Check sheet for the modelled part. Datum: model origin and axes. Units: mm. A direction names the side the tool comes from. Give positions to 0.01 mm unless a question says otherwise; leave off trailing zeros. Order: outer loops, then holes, each group sorted by start corner. A loop starts at its lowest first (then second) coordinate and runs counter-clockwise, first axis right, second up.
Item 1: Sectioned sample at D-D on y = 24. Record the boundary of the cut face in (x, z), and give its area (3 significant figures).
Item 2: Sectioned sample at B-B on x = 0. Record the boundary of the cut face in (y, z).
Item 3: Release check for a two-part mould opening along Z. For faces 1 (the cylindrical face through (-45.72, 22.32, -45.49)), 2 (the flat face through (44, 22, 0)), 3 (the flat face through (45, 35, 0)) record: released by +Z, released by -Z, zero draft, split by the parting line, or undercut.
Item 4: Sectioned sample at C-C on z = 17.5. Record the boundary of the cut face in (x, y).
Item 5: Sectioned sample at A-A on y = -3. Count the separate pieces of the cut face and the enclosed holes in it, and give its area (3 significant figures).
Item 6: Access from +Z, -Z, +X, -X, +Y, -Y to the whole of each face (thin tool, end or side, straight path). Record for faces 4 (the flat face through (73, -10, 6)), 5 (the flat face through (84.064, 0.14, 39.556)), 6 (the cylindrical face through (41.434, 22.325, -41.294)), 7 (the cylindrical face through (45.49, 22.32, -45.72)).
Item 7: Material ranges on line 1 along X through (y, z) = (2, -65); line 2 along X through (y, z) = (-7.8, 0); line 3 along Z through (x, y) = (-22, 26), recorded low to high.
Item 8: Gauge pin test, flat ends, axial feed: P1, Ø4, axis at y = 13, z = -57, coming from the +X side; P2, Ø6, axis at x = -65.5, z = 20.5, coming from the +Y side; P3, Ø1, axis at y = 20.5, z = 19.5, coming from the -X side; P4, Ø1.5, axis at x = 62.5, z = 17.5, coming from the -Y side. Record the tip position at first contact, or that the pin passes through.
from build123d import *

# Parameters (mm, degrees)
BASE_FLANGE_SKETCH_R      = 6.5
BASE_FLANGE_DEPTH         = 10
SQUARE_BOSS_DEPTH         = 25
BOSS_POCKET_DEPTH         = 130.711217711
BOSS_POCKET_DEPTH_BACK    = 130.711217711
BOSS_POCKET_SKETCH_R      = 9.473120825
RECESS_CUT_3MM_DEPTH      = 136
RECESS_CUT_3MM_DEPTH_BACK = 3
RECESS_SKETCH_R           = 72.5
RECESS_SKETCH_R_2         = 52.5


with BuildPart() as part:
    # Base Flange Sketch → Base Flange (new, symmetric)
    with BuildSketch(Plane(origin=(0, 0, 0), x_dir=(1, 0, 0), z_dir=(0, 1, 0))):
        with BuildLine():
            Line((-89.148145657, 58.529523872), (-78.836109635, 20.044481509))
            ThreePointArc((-78.836109635, 20.044481509), (-78.436026062, 17.398303615), (-78.632364827, 14.72926345))
            ThreePointArc((-78.632364827, 14.72926345), (-80, 0), (-78.632364827, -14.72926345))
            ThreePointArc((-78.632364827, -14.72926345), (-78.436026062, -17.398303615), (-78.836109635, -20.044481509))
            Line((-78.836109635, -20.044481509), (-89.148145657, -58.529523872))
            ThreePointArc((-89.148145657, -58.529523872), (-82.67766953, -82.67766953), (-58.529523872, -89.148145657))
            Line((-58.529523872, -89.148145657), (-20.044481509, -78.836109635))
            ThreePointArc((-20.044481509, -78.836109635), (-17.398303615, -78.436026062), (-14.72926345, -78.632364827))
            ThreePointArc((-14.72926345, -78.632364827), (0, -80), (14.72926345, -78.632364827))
            ThreePointArc((14.72926345, -78.632364827), (17.398303615, -78.436026062), (20.044481509, -78.836109635))
            Line((20.044481509, -78.836109635), (58.529523872, -89.148145657))
            ThreePointArc((58.529523872, -89.148145657), (82.67766953, -82.67766953), (89.148145657, -58.529523872))
            Line((89.148145657, -58.529523872), (78.836109635, -20.044481509))
            ThreePointArc((78.836109635, -20.044481509), (78.436026062, -17.398303615), (78.632364827, -14.72926345))
            ThreePointArc((78.632364827, -14.72926345), (80, 0), (78.632364827, 14.72926345))
            ThreePointArc((78.632364827, 14.72926345), (78.436026062, 17.398303615), (78.836109635, 20.044481509))
            Line((78.836109635, 20.044481509), (89.148145657, 58.529523872))
            ThreePointArc((89.148145657, 58.529523872), (82.67766953, 82.67766953), (58.529523872, 89.148145657))
            Line((58.529523872, 89.148145657), (20.044481509, 78.836109635))
            ThreePointArc((20.044481509, 78.836109635), (17.398303615, 78.436026062), (14.72926345, 78.632364827))
            ThreePointArc((14.72926345, 78.632364827), (0, 80), (-14.72926345, 78.632364827))
            ThreePointArc((-14.72926345, 78.632364827), (-17.398303615, 78.436026062), (-20.044481509, 78.836109635))
            Line((-20.044481509, 78.836109635), (-58.529523872, 89.148145657))
            ThreePointArc((-58.529523872, 89.148145657), (-82.67766953, 82.67766953), (-89.148145657, 58.529523872))
        make_face()
        with Locations(Location((-65, 65, 0), (0, 0, 270))):
            Circle(BASE_FLANGE_SKETCH_R, mode=Mode.SUBTRACT)
        with Locations(Location((65, 65, 0), (0, 0, 270))):
            Circle(BASE_FLANGE_SKETCH_R, mode=Mode.SUBTRACT)
        with Locations(Location((65, -65, 0), (0, 0, 270))):
            Circle(BASE_FLANGE_SKETCH_R, mode=Mode.SUBTRACT)
        with Locations(Location((-65, -65, 0), (0, 0, 270))):
            Circle(BASE_FLANGE_SKETCH_R, mode=Mode.SUBTRACT)
    extrude(amount=BASE_FLANGE_DEPTH, both=True)

    # Square Boss Sketch → Square Boss (add)
    with BuildSketch(Plane(origin=(0, 10, 0), x_dir=(1, 0, 0), z_dir=(0, 1, 0))):
        with BuildLine():
            Line((-35, 50), (35, 50))
            ThreePointArc((35, 50), (45.606601718, 45.606601718), (50, 35))
            Line((50, 35), (50, -35))
            ThreePointArc((50, -35), (45.606601718, -45.606601718), (35, -50))
            Line((35, -50), (-35, -50))
            ThreePointArc((-35, -50), (-45.606601718, -45.606601718), (-50, -35))
            Line((-50, -35), (-50, 35))
            ThreePointArc((-50, 35), (-45.606601718, 45.606601718), (-35, 50))
        make_face()
        with BuildLine():
            ThreePointArc((-35, 44), (-41.363961031, 41.363961031), (-44, 35))
            Line((-44, 35), (-44, -35))
            ThreePointArc((-44, -35), (-41.363961031, -41.363961031), (-35, -44))
            Line((-35, -44), (35, -44))
            ThreePointArc((35, -44), (41.363961031, -41.363961031), (44, -35))
            Line((44, -35), (44, 35))
            ThreePointArc((44, 35), (41.363961031, 41.363961031), (35, 44))
            Line((35, 44), (-35, 44))
        make_face(mode=Mode.SUBTRACT)
    extrude(amount=SQUARE_BOSS_DEPTH)

    # Boss Pocket Sketch → Boss Pocket (cut, two sides: drawn at the far end of the back side and taken through both)
    with BuildSketch(Plane(origin=(0, 10, 0), x_dir=(1, 0, 0), z_dir=(0, 1, 0)).offset(-BOSS_POCKET_DEPTH_BACK)):
        with Locations(Location((-22, -22, 0), (0, 0, 270))):
            Circle(BOSS_POCKET_SKETCH_R)
        with Locations(Location((22, -22, 0), (0, 0, 270))):
            Circle(BOSS_POCKET_SKETCH_R)
        with Locations(Location((22, 22, 0), (0, 0, 270))):
            Circle(BOSS_POCKET_SKETCH_R)
        with Locations(Location((-22, 22, 0), (0, 0, 270))):
            Circle(BOSS_POCKET_SKETCH_R)
    extrude(amount=BOSS_POCKET_DEPTH + BOSS_POCKET_DEPTH_BACK, mode=Mode.SUBTRACT)

    # Recess Sketch → Recess Cut 3mm (cut, two sides: drawn at the far end of the back side and taken through both)
    with BuildSketch(Plane.XZ.offset(10).offset(-RECESS_CUT_3MM_DEPTH_BACK)):
        with Locations(Location((0, 0, 0), (0, 0, 270))):
            Circle(RECESS_SKETCH_R)
        with Locations(Location((0, 0, 0), (0, 0, 270))):
            Circle(RECESS_SKETCH_R_2, mode=Mode.SUBTRACT)
    extrude(amount=RECESS_CUT_3MM_DEPTH + RECESS_CUT_3MM_DEPTH_BACK, mode=Mode.SUBTRACT)


solid = part.part
Report:
1. outline: (-50, -35) arc R15 ccw to (-35, -50) - (35, -50) arc R15 ccw to (50, -35) - (50, 35) arc R15 ccw to (35, 50) - (-35, 50) arc R15 ccw to (-50, 35) - close; hole (-44, -35) arc R9 ccw to (-35, -44) - (35, -44) arc R9 ccw to (44, -35) - (44, 35) arc R9 ccw to (35, 44) - (-35, 44) arc R9 ccw to (-44, 35) - close
1. area: 2,130 mm2
2. outline: (-10, -80) - (10, -80) - (10, -50) - (35, -50) - (35, -44) - (10, -44) - (10, 44) - (35, 44) - (35, 50) - (10, 50) - (10, 80) - (-10, 80) - (-10, 72.5) - (-7, 72.5) - (-7, 52.5) - (-10, 52.5) - (-10, -52.5) - (-7, -52.5) - (-7, -72.5) - (-10, -72.5) - close
3. face 1: released by -Z
3. face 2: undercut
3. face 3: zero draft
4. outline: (-78.44, -10) - (-70.36, -10) - (-70.36, -7) - (-49.5, -7) - (-49.5, -10) - (-30.34, -10) - (-30.34, 10) - (-44, 10) - (-44, 35) - (-50, 35) - (-50, 10) - (-78.44, 10) - close; (-13.66, -10) - (13.66, -10) - (13.66, 10) - (-13.66, 10) - close; (30.34, -10) - (49.5, -10) - (49.5, -7) - (70.36, -7) - (70.36, -10) - (78.44, -10) - (78.44, 10) - (50, 10) - (50, 35) - (44, 35) - (44, 10) - (30.34, 10) - close
5. separate pieces: 1
5. enclosed holes: 8
5. area: 26,600 mm2
6. face 4: +Z, -Z, +X, -X, -Y
6. face 5: +X, +Y, -Y
6. face 6: +Y
6. face 7: -Z, +X, +Y
7. line 1: x = -90 to -71.5, -58.5 to 58.5, 71.5 to 90
7. line 2: x = -80 to -72.5, -52.5 to 52.5, 72.5 to 80
7. line 3: z = -50 to -44, 44 to 50
8. P1: passes through
8. P2: stops at y = 10
8. P3: stops at x = -50
8. P4: stops at y = -7
